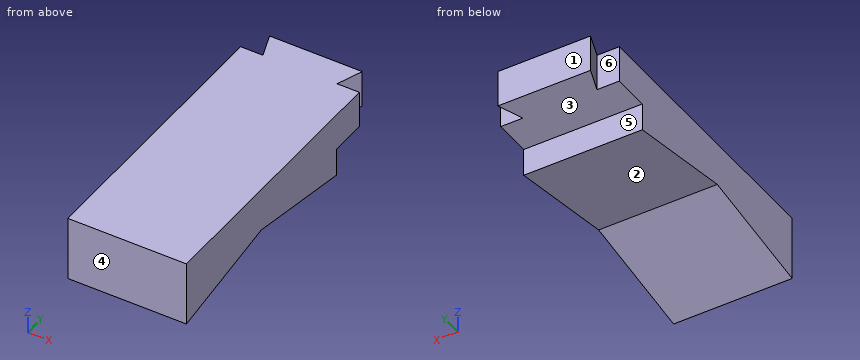
```python
from build123d import *

# Parameters (mm, degrees)
BOSS_EXTRUDE1_DEPTH = 20
BOSS_EXTRUDE2_DEPTH = 64


with BuildPart() as part:
    # Sketch1 → Boss-Extrude1 (new body)
    with BuildSketch(Plane.XY):
        Polygon((-27.262159038, -0.780894157), (-27.262159038, -150.780894157), (36.737840962, -150.780894157), (36.737840962, -0.780894157), (24.737840962, -0.780894157), (29.737840962, 12.95649294), (-20.262159038, 12.95649294), (-15.262159038, -0.780894157), align=None)
    extrude(amount=BOSS_EXTRUDE1_DEPTH)

    # Sketch2 → Boss-Extrude2 (add)
    with BuildSketch(Plane(origin=(36.737840962, 0, 0), x_dir=(0, 0, -1), z_dir=(1, 0, 0))):
        Polygon((0, -150.780894157), (15, -150.780894157), (3.538746274, -85.783666039), (15, -20.780894157), (0, -20.780894157), align=None)
    extrude(amount=-BOSS_EXTRUDE2_DEPTH)


solid = part.part
```
The model under review builds one solid part; all positions refer to its coordinate system, in mm. Face numbers are marked on the shaded views. A direction names the side the tool comes from. Round coordinates to 2 decimals unless told otherwise and drop trailing zeros. Write each loop counter-clockwise with the first axis right and the second up, starting at its lowest first coordinate (ties: lowest second). Pieces come first, ordered by that corner, then holes. Notation, with made-up numbers: M 20,2 L 33,2 A14 cw 33,11 Z; hole C 86.25,-20 d3. An arc over 180 degrees is marked long. Use CSV: the item, a comma, the result in double quotes. Start each with the question number.
(1) Clearance check with flat-ended pins moving along their axes: P1, Ø7.5, axis at x = 2, z = -9, coming from the +Y side; P2, Ø10, axis at x = -8.5, y = -12, coming from the -Z side. State where each tip first meets the part, or that it passes through.
(2) We need section B-B, the plane z = 18.5. State the section outline as (x, y) points, then the cut area to 3 significant figures.
(3) For line 1 along Y through (x, z) = (-8, -1); line 2 along Z through (x, y) = (23, -6); line 3 along Y through (x, z) = (31, 8), list the stretches that pass through material, from the lowest coordinate up.
(4) We need section C-C, the plane x = 0. State the section outline as (y, z) points.
(5) The part is to be moulded in two halves that separate along Y. For the marked faces 4, 5 and 6, say which applies: +Y half, -Y half, draft (parallel to the pull), parting line (faces both ways), or undercut.
(6) We need section A-A, the plane x = -18.5. State the section outline as (y, z) points (1 decimal).
(7) We need section D-D, the plane z = -7. State the section outline as (x, y) points.
(8) Tool access review of the marked faces 1, 2 and 3: name each direction out of +Z, -Z, +X, -X, +Y, -Y from which nothing blocks a thin tool from reaching the whole face with its end or side.
Findings:
1,P1,"y = -20.78"
1,P2,"z = 0"
2,outline,"M -27.26,-150.78 L 36.74,-150.78 L 36.74,-0.78 L 24.74,-0.78 L 29.74,12.96 L -20.26,12.96 L -15.26,-0.78 L -27.26,-0.78 Z"
2,area,"10,200 mm^2"
3,line 1,"-150.78 to -20.78"
3,line 2,"0 to 20"
3,line 3,"-150.78 to -0.78"
4,outline,"M -150.78,-15 L -85.78,-3.54 L -20.78,-15 L -20.78,0 L 12.96,0 L 12.96,20 L -150.78,20 Z"
5,face 4,"-Y half"
5,face 5,"+Y half"
5,face 6,"undercut"
6,outline,"M -150.8,-15 L -85.8,-3.5 L -20.8,-15 L -20.8,0 L -0.8,0 L -0.8,20 L -150.8,20 Z; M 8.1,0 L 13,0 L 13,20 L 8.1,20 Z"
7,outline,"M -27.26,-150.78 L 36.74,-150.78 L 36.74,-105.41 L -27.26,-105.41 Z; M -27.26,-66.15 L 36.74,-66.15 L 36.74,-20.78 L -27.26,-20.78 Z"
8,face 1,"+Z, -Z, +X, -X, +Y"
8,face 2,"-Z, +X, -X"
8,face 3,"-Z, +X, -X, +Y"
